from build123d import *

# Parameters (mm, degrees)
BASE_BODY_DEPTH          = 20
HUB_BOSS_SKETCH_R        = 20
HUB_BOSS_DEPTH           = 30
HUB_BORE_SKETCH_R        = 10
HUB_BORE_20_DEPTH        = 205.694894905
FOOT_BLOCK_SKETCH_R      = 25
FOOT_BLOCK_DEPTH         = 35
HINGE_PLATE_DEPTH        = 20
PLATE_STIFFENER_SKETCH_R = 15
PLATE_STIFFENER_DEPTH    = 20
PIN_BOSS_SKETCH_W        = 60
PIN_BOSS_SKETCH_H        = 60
PIN_BOSS_DEPTH           = 20
HUB_FILLET_R5_R          = 5
FOOT_BLOCK_FILLET_R10_R  = 10
HINGE_PLATE_FILLET_R20_R = 20


with BuildPart() as part:
    # Base Profile Sketch → Base Body (new body)
    with BuildSketch(Plane(origin=(0, 0, 0), x_dir=(0, 0, -1), z_dir=(1, 0, 0))):
        with BuildLine():
            Line((45, 50), (-45, 50))
            Line((-45, 50), (-109.504258609, 28.45468447))
            ThreePointArc((-109.504258609, 28.45468447), (-130, 0), (-109.504258609, -28.45468447))
            Line((-109.504258609, -28.45468447), (-58.663827594, -45.436092388))
            ThreePointArc((-58.663827594, -45.436092388), (-48.771576661, -52.716644423), (-45, -64.405882035))
            Line((-45, -64.405882035), (-45, -150))
            Line((-45, -150), (45, -150))
            Line((45, -150), (45, -64.405882035))
            ThreePointArc((45, -64.405882035), (48.771576661, -52.716644423), (58.663827594, -45.436092388))
            Line((58.663827594, -45.436092388), (109.504258609, -28.45468447))
            ThreePointArc((109.504258609, -28.45468447), (130, 0), (109.504258609, 28.45468447))
            Line((109.504258609, 28.45468447), (45, 50))
        make_face()
    extrude(amount=BASE_BODY_DEPTH)

    # Hub Boss Sketch → Hub Boss (add)
    with BuildSketch(Plane.ZY):
        with Locations(Location((-100, 0, 0), (0, 0, 180))):
            Circle(HUB_BOSS_SKETCH_R)
        with Locations(Location((100, 0, 0), (0, 0, 180))):
            Circle(HUB_BOSS_SKETCH_R)
    extrude(amount=HUB_BOSS_DEPTH)

    # Hub Bore Sketch → Hub Bore Ø20 (cut, through all)
    with BuildSketch(Plane.ZY.offset(30)):
        with Locations((-100, 0)):
            Circle(HUB_BORE_SKETCH_R)
        with Locations((100, 0)):
            Circle(HUB_BORE_SKETCH_R)
    extrude(amount=-HUB_BORE_20_DEPTH, mode=Mode.SUBTRACT)

    # Foot Block Sketch → Foot Block (add, symmetric)
    with BuildSketch(Plane(origin=(0, 0, 0), x_dir=(1, 0, 0), z_dir=(0, 1, 0))):
        with BuildLine():
            Line((-57, 43), (0, 43))
            Line((0, 43), (0, -43))
            Line((0, -43), (-57, -43))
            ThreePointArc((-57, -43), (-100, 0), (-57, 43))
        make_face()
        with Locations(Location((-57, 0, 0), (0, 0, 270))):
            Circle(FOOT_BLOCK_SKETCH_R, mode=Mode.SUBTRACT)
    extrude(amount=FOOT_BLOCK_DEPTH, both=True)

    # Hinge Plate Sketch → Hinge Plate (add)
    with BuildSketch(Plane.XZ.offset(150)):
        Polygon((20, 0), (20, 80), (-40, 80), (-40, 33), (-115, 33), (-115, -33), (-40, -33), (-40, -80), (20, -80), align=None)
    extrude(amount=HINGE_PLATE_DEPTH)

    # Plate Stiffener Sketch → Plate Stiffener (add)
    with BuildSketch(Plane.ZY.offset(115)):
        with BuildLine():
            Line((-33, -150), (33, -150))
            Line((33, -150), (33, -227))
            ThreePointArc((33, -227), (0, -260), (-33, -227))
            Line((-33, -227), (-33, -150))
        make_face()
        with Locations((0, -227)):
            Circle(PLATE_STIFFENER_SKETCH_R, mode=Mode.SUBTRACT)
    extrude(amount=-PLATE_STIFFENER_DEPTH)

    # Pin Boss Sketch → Pin Boss (add)
    with BuildSketch(Plane.XY.offset(80)):
        with Locations((-10, -180)):
            Rectangle(PIN_BOSS_SKETCH_W, PIN_BOSS_SKETCH_H)
    pin_boss = extrude(amount=-PIN_BOSS_DEPTH)

    # Pin Boss Mirror: Pin Boss across plane
    add(pin_boss.mirror(Plane.XY))

    # Hub Fillet R5
    hub_fillet_r5_edges = [part.edges().sort_by_distance(p)[0] for p in [
        (0, 0, -80),
        (0, 0, 120),
    ]]
    fillet(hub_fillet_r5_edges, radius=HUB_FILLET_R5_R)

    # Foot Block Fillet R10
    foot_block_fillet_r10_edges = [part.edges().sort_by_distance(p)[0] for p in [
        (0, 0, 43),
        (0, 0, -43),
    ]]
    fillet(foot_block_fillet_r10_edges, radius=FOOT_BLOCK_FILLET_R10_R)

    # Hinge Plate Fillet R20
    hinge_plate_fillet_r20_edges = [part.edges().sort_by_distance(p)[0] for p in [
        (10, -150, -45),
        (10, -150, 45),
    ]]
    fillet(hinge_plate_fillet_r20_edges, radius=HINGE_PLATE_FILLET_R20_R)


solid = part.part
Work out the finished part from the listing and answer in its coordinate system (mm). A direction names the side the tool comes from. Coordinates: 2 decimals unless noted, no trailing zeros. Write each loop counter-clockwise with the first axis right and the second up, starting at its lowest first coordinate (ties: lowest second). Pieces come first, ordered by that corner, then holes. Notation, with made-up numbers: M 21.25,60.25 L 39.25,60.25 A23 cw 39.25,93.25 Z; hole C -27,-12 d8. An arc over 180 degrees is marked long. Answer as CSV lines item,"result". Start each with the question number.
Item 1: Flat-ended cylindrical pins translate along their axes: P1, Ø12, axis at x = 3.5, y = -149.5, coming from the +Z side; P2, Ø12, axis at y = 0, z = 100, coming from the +X side; P3, Ø12, axis at x = -7.5, z = -98, coming from the -Y side; P4, Ø20, axis at y = 8, z = 107, coming from the -X side. Find the tip coordinate at first contact, or state that the pin passes through.
Item 2: Determine the mould class of faces 1 (the face through (9.86, -37.064, -83.728)), 2 (the face through (-5, 0, -110)), 3 (the face through (-27, 35, -1)) for opening direction Z: released by +Z, released by -Z, zero draft, split by the parting line, or undercut.
Item 3: Section B-B on x = -18.5 is taken. Write down the section's boundary in (y, z), and give its area (3 significant figures).
Item 4: A tool of negligible diameter and unlimited length cuts with its end or side. For faces 4 (the face through (-2.85, -0.49, -46.01)), 5 (the face through (10, -97, 45)), 6 (the face through (9.86, -52.86, -48.67)), 7 (the face through (-26, -170, 1)), from which of +Z, -Z, +X, -X, +Y, -Y can it reach the whole face along a straight path? Write none if from no direction.
Item 5: Section A-A on y = 0 is taken. Give the number of separate pieces and of enclosed holes in the cut face, and give its area (3 significant figures).
Item 6: Section D-D on y = -180.5 is taken. Write down the section's boundary in (x, z), and give its area (3 significant figures).
Item 7: Consider L1, parallel to Y at x = -21, z = -16; L2, parallel to Y at x = -17, z = -100; L3, parallel to X at y = -11, z = 0. Determine where each line is inside the solid, lowest interval first.
Item 8: Section C-C on z = 0 is taken. Write down the section's boundary in (x, y).
Checks:
1,P1,"stops at z = 80"
1,P2,"passes through"
1,P3,"stops at y = -21.36"
1,P4,"stops at x = -30"
2,face 1,"released by -Z"
2,face 2,"undercut"
2,face 3,"zero draft"
3,outline,"M -210,-80 L -150,-80 L -150,80 L -210,80 L -210,60 L -170,60 L -170,-60 L -210,-60 Z; M -35,-43 L 35,-43 L 35,43 L -35,43 Z; C 0,-100 d40; C 0,100 d40; hole C 0,-100 d20; hole C 0,100 d20"
3,area,"12,700 mm²"
4,face 4,"-X, +Y"
4,face 5,"+Z, +X, -X"
4,face 6,"-Z, +X, -X"
4,face 7,"+X, -Y"
5,separate pieces,"3"
5,enclosed holes,"1"
5,area,"11,500 mm²"
6,outline,"M -115,-33 L -95,-33 L -95,33 L -115,33 Z; M -40,-80 L 20,-80 L 20,-60 L -40,-60 Z; M -40,60 L 20,60 L 20,80 L -40,80 Z"
6,area,"3,720 mm²"
7,L1,"y = -170 to -150, -35 to 35"
7,L2,"y = -20 to -10, 10 to 20"
7,L3,"x = -100 to -82, -32 to 20"
8,outline,"M -115,-260 L -95,-260 L -95,-242 L -115,-242 Z; M -115,-212 L -95,-212 L -95,-170 L 20,-170 L 20,50 L 0,50 L 0,35 L -32,35 L -32,-35 L 0,-35 L 0,-150 L -115,-150 Z; M -100,-35 L -82,-35 L -82,35 L -100,35 Z"
